from build123d import *

# Parameters (mm, degrees)
CHAMFER1_SIZE  = 5
CHAMFER1_SIZE2 = 0.881634904
CHAMFER2_SIZE  = 1


with BuildPart() as part:
    # Sketch3 → Revolve1 (revolve)
    with BuildSketch(Plane(origin=(0, 0, 0), x_dir=(0, 0, -1), z_dir=(1, 0, 0)), mode=Mode.PRIVATE) as revolve1_sk:
        Polygon((-325, 25), (629, 25), (629, 17.799192231), (630.760753628, 15.700807769), (630.760753628, 8.5), (633.5, 8.5), (633.5, 7.5), (644.5, 7.5), (644.5, 0), (-340.5, 0), (-340.5, 7.5), (-329.5, 7.5), (-329.5, 8.5), (-326.760753628, 8.5), (-326.760753628, 15.700807769), (-325, 17.799192231), align=None)
    revolve(revolve1_sk.sketch.rotate(Axis((0, 0, 340.5), (0, 0, -1)), 90), axis=Axis((0, 0, 340.5), (0, 0, -1)))

    # Chamfer1
    chamfer1_edges = [part.edges().sort_by_distance(p)[0] for p in [
        (-25, 0, -629),
        (-25, 0, 325),
    ]]
    chamfer1_side = [part.faces().sort_by_distance(p)[0] for p in [
        (-25, 0, -152),
    ]]
    chamfer(chamfer1_edges, length=CHAMFER1_SIZE, length2=CHAMFER1_SIZE2, reference=chamfer1_side[0])

    # Chamfer2
    chamfer2_edges = [part.edges().sort_by_distance(p)[0] for p in [
        (-7.5, 0, 340.5),
        (-7.5, 0, -644.5),
    ]]
    chamfer(chamfer2_edges, length=CHAMFER2_SIZE)


solid = part.part
Build history of the part. All positions in model axes, mm. A direction names the side the tool comes from. Give positions to 0.01 mm unless a question says otherwise; leave off trailing zeros. Loops run counter-clockwise (first coordinate to the right, second up) from the corner with the lowest first, then second, coordinate; pieces in that order, holes last. Notation, with made-up numbers: (21.25, 61.5) -> (66.25, 61.5) arc R30 cw to (66.25, 100.5) -> close; hole circle Ø3 at (80, 4). An arc over 180 degrees is marked (long way). Answer in a Markdown table with one row per item.
Item 1: Slice it at A-A on z = 3. Write the cut outline in (x, y), plus the area to 3 significant figures.
Findings below:
| item | result |
|---|---|
| outline | circle Ø50 at (0, 0) |
| area | 1,960 mm² |
Item 2: Probe line 1 along Z through (x, y) = (-13.5, 19.5); line 2 along X through (y, z) = (6, 57); line 3 along Z through (x, y) = (-7, -11.5). List the from-to ranges inside material, lowest first. Write a range as [from, to].
Findings below:
| item | result |
|---|---|
| line 1 | z = [-629, 325] |
| line 2 | x = [-24.27, 24.27] |
| line 3 | z = [-630.76, 326.76] |
Item 3: Flat gauge pins, fed straight in: P1, Ø12, axis at y = -14, z = 106, coming from the -X side; P2, Ø12, axis at x = 17.5, y = -15.5, coming from the +Z side; P3, Ø10, axis at y = 8, z = -130, coming from the +X side. Where does each tip first touch, or does it go through?
Findings below:
| item | result |
|---|---|
| P1 | stops at x = -23.69 |
| P2 | stops at z = 325.35 |
| P3 | stops at x = 24.82 |
Item 4: Tool access for faces 1 (the flat face through (-2, 18, -629)), 2 (the cylindrical face through (23.846, -7.509, -158.608)), 3 (the cylindrical face through (-1.107, -8.428, 328.111)): list every direction of +Z, -Z, +X, -X, +Y, -Y with a clear straight run to the whole face (end or side of a thin tool).
Findings below:
| item | result |
|---|---|
| face 1 | -Z |
| face 2 | +Z, -Z |
| face 3 | +Z |
